Part model, mm, in its own coordinate system. Face numbers are marked on the shaded views. A direction names the side the tool comes from. Coordinates: 2 decimals unless noted, no trailing zeros. Loops run counter-clockwise (first coordinate to the right, second up) from the corner with the lowest first, then second, coordinate; pieces in that order, holes last. Notation, with made-up numbers: (25, 77.5) - (79, 77.5) arc R31 cw to (79, 113.5) - close; hole circle Ø9 at (89.25, 76.5). An arc over 180 degrees is marked (long way). Answer as CSV lines item,"result".
from build123d import *

# Parameters (mm, degrees)
EXTRUDE_1_DEPTH = 10


with BuildPart() as part:
    # 草图1 → 凸台-拉伸1 (new body)
    with BuildSketch(Plane.XY):
        with BuildLine():
            Line((-37.5, 54.4), (-37.5, -70.6))
            ThreePointArc((-37.5, -70.6), (-36.035533906, -74.135533906), (-32.5, -75.6))
            Line((-32.5, -75.6), (32.5, -75.6))
            ThreePointArc((32.5, -75.6), (36.035533906, -74.135533906), (37.5, -70.6))
            Line((37.5, -70.6), (37.5, 54.4))
            Line((37.5, 54.4), (-37.5, 54.4))
        make_face()
        with BuildLine():
            Line((-9.03462289, -27), (-9.029321888, -26.984157939))
            ThreePointArc((-9.029321888, -26.984157939), (-2.503961636, -19.764527679), (-9.5, -13))
            Line((-9.5, -13), (-25.5, -13))
            ThreePointArc((-25.5, -13), (-32.5, -20), (-25.5, -27))
            Line((-25.5, -27), (-9.03462289, -27))
        make_face(mode=Mode.SUBTRACT)
        with BuildLine():
            ThreePointArc((18.5, -28), (25.5, -35), (32.5, -28))
            Line((32.5, -28), (32.5, -12))
            ThreePointArc((32.5, -12), (25.5, -5), (18.5, -12))
            Line((18.5, -12), (18.5, -28))
        make_face(mode=Mode.SUBTRACT)
    extrude(amount=EXTRUDE_1_DEPTH)


solid = part.part
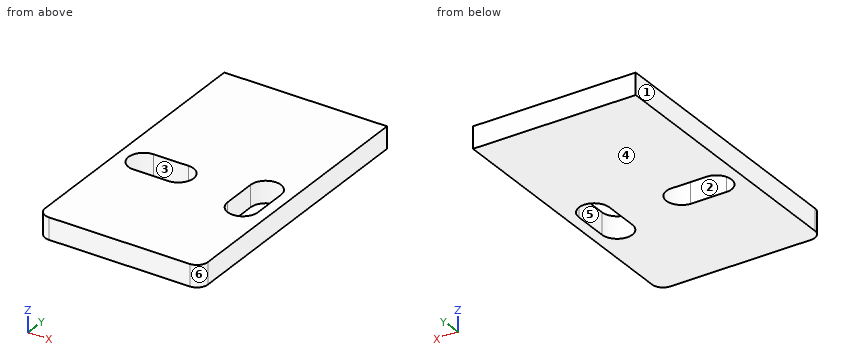
Q1. Saw through at D-D (x = 25.5). Give the cut face in (y, z), then the cut area to 3 significant figures.
Results:
outline,"(-75.6, 0) - (-35, 0) - (-35, 10) - (-75.6, 10) - close; (-5, 0) - (54.4, 0) - (54.4, 10) - (-5, 10) - close"
area,"1,000 mm^2"
Q2. Wall check: L1, parallel to Y at x = -14, z = 6; L2, parallel to X at y = -12.5, z = 1.5; L3, parallel to Y at x = -33, z = 2. Give the ranges that are in metal, low to high.
Results:
L1,"y = -75.6 to -27, -13 to 54.4"
L2,"x = -37.5 to 18.5, 32.5 to 37.5"
L3,"y = -75.57 to 54.4"
Q3. Saw through at B-B (x = -12). Give the cut face in (y, z).
Results:
outline,"(-75.6, 0) - (-27, 0) - (-27, 10) - (-75.6, 10) - close; (-13, 0) - (54.4, 0) - (54.4, 10) - (-13, 10) - close"
Q4. Two-plate mould, pull along X, no slides. Class the marked faces 1, 2, 3 and 4: released by +X, released by -X, zero draft, split by the parting line, or undercut.
Results:
face 1,"released by -X"
face 2,"undercut"
face 3,"undercut"
face 4,"zero draft"
Q5. Which spindle directions (+Z, -Z, +X, -X, +Y, -Y) get a long thin tool onto all of the face, cutting with end or side? Do the marked faces 5 and 6. Say none if no direction does.
Results:
face 5,"+Z, -Z"
face 6,"+Z, -Z, +X, -Y"
Q6. Saw through at C-C (z = 4.5). Count the separate pieces of the cut face and the enclosed holes in it, then the cut area to 3 significant figures.
Results:
separate pieces,"1"
enclosed holes,"2"
area,"8,980 mm^2"
Q7. Saw through at A-A (y = -20). Give the cut face in (x, z).
Results:
outline,"(-37.5, 0) - (-32.5, 0) - (-32.5, 10) - (-37.5, 10) - close; (-2.5, 0) - (18.5, 0) - (18.5, 10) - (-2.5, 10) - close; (32.5, 0) - (37.5, 0) - (37.5, 10) - (32.5, 10) - close"
